from build123d import *

# Parameters (mm, degrees)
SKETCH1_W                = 37
SKETCH1_H                = 30
SKETCH1_W_2              = 20
SKETCH1_H_2              = 20
M4_CLEARANCE_HOLE1_D     = 4.5
M4_CLEARANCE_HOLE1_DEPTH = 30
M4_CLEARANCE_HOLE2_D     = 4.5


with BuildPart() as part:
    # Sweep1: sweep along a path in Sketch2
    with BuildLine(Plane.XY) as sweep1_path:
        Line((0, 0), (75, 0))
        ThreePointArc((75, 0), (115, 40), (75, 80))
        Line((75, 80), (-100, 80))
    # Sketch1 → Sweep1 (sweep)
    with BuildSketch(Plane(origin=(0, 0, 0), x_dir=(0, 0, -1), z_dir=(1, 0, 0))):
        Rectangle(SKETCH1_W, SKETCH1_H)
        Rectangle(SKETCH1_W_2, SKETCH1_H_2, mode=Mode.SUBTRACT)
    sweep(path=sweep1_path.line)

    # M4 Clearance Hole1
    with Locations(Plane(origin=(0, 15, 0), x_dir=(1, 0, 0), z_dir=(0, 1, 0))):
        with Locations((8.5, 14.5), (8.5, -14.5)):
            Hole(M4_CLEARANCE_HOLE1_D / 2, depth=M4_CLEARANCE_HOLE1_DEPTH)

    # M4 Clearance Hole2 (through all)
    with Locations(Plane(origin=(0, 95, 0), x_dir=(1, 0, 0), z_dir=(0, 1, 0))):
        with Locations((-91.5, -14.5), (-91.5, 14.5)):
            Hole(M4_CLEARANCE_HOLE2_D / 2)


solid = part.part
Verification items for the finished model (mm, model axes). A direction names the side the tool comes from. Coordinates: 2 decimals unless noted, no trailing zeros. Order: outer loops, then holes, each group sorted by start corner. A loop starts at its lowest first (then second) coordinate and runs counter-clockwise, first axis right, second up. Notation, with made-up numbers: M -12,83 L 0,83 A24 cw 0,95 Z; hole C -34,-7 d3. An arc over 180 degrees is marked long. Return JSON: item names as keys, results as strings.
1) Access from +Z, -Z, +X, -X, +Y, -Y to the whole of each face (thin tool, end or side, straight path). Record for faces 5 (the cylindrical face through (10.286, -0.21, -13.131)), 6 (the flat face through (-14, 65, 0)), 7 (the flat face through (38, 73, 10)), 8 (the flat face through (38, 10, 0)).
Answer list:
{"face 5": "-Y", "face 6": "+Z, -Z, -X", "face 7": "none", "face 8": "-X"}
2) Thickness scan on L1, parallel to Y at x = 41.5, z = 8; L2, parallel to Z at x = 8, y = -3; L3, parallel to Z at x = 104, y = 59.5. Record the ranges inside material, lowest first. Write a range as [from, to].
Answer list:
{"L1": "[-15, -10], [10, 15], [65, 70], [90, 95]", "L2": "[-18.5, -16.69], [-12.31, -10], [10, 12.31], [16.69, 18.5]", "L3": "[-18.5, -10], [10, 18.5]"}
3) Cross-section at B-B, the plane z = 14.5. Record the boundary of the cut face in (x, y).
Answer list:
{"outline": "M -100,65 L -93.75,65 L -93.75,95 L -100,95 Z; M -89.25,65 L 75,65 A25 cw 75,15 L 10.75,15 L 10.75,-15 L 75,-15 A55 ccw 75,95 L -89.25,95 Z; M 0,-15 L 6.25,-15 L 6.25,15 L 0,15 Z"}
4) Cross-section at C-C, the plane x = 8.5. Record the boundary of the cut face in (y, z).
Answer list:
{"outline": "M -15,-18.5 L 15,-18.5 L 15,-16.75 L -15,-16.75 Z; M -15,-12.25 L 15,-12.25 L 15,12.25 L -15,12.25 Z; M -15,16.75 L 15,16.75 L 15,18.5 L -15,18.5 Z; M 65,-18.5 L 95,-18.5 L 95,18.5 L 65,18.5 Z; hole M -10,-10 L 10,-10 L 10,10 L -10,10 Z; hole M 70,-10 L 90,-10 L 90,10 L 70,10 Z"}
5) Cross-section at D-D, the plane z = -3.5. Record the boundary of the cut face in (x, y).
Answer list:
{"outline": "M -100,65 L 75,65 A25 cw 75,15 L 0,15 L 0,10 L 75,10 A30 ccw 75,70 L -100,70 Z; M -100,90 L 75,90 A50 cw 75,-10 L 0,-10 L 0,-15 L 75,-15 A55 ccw 75,95 L -100,95 Z"}
6) Release check for a two-part mould opening along Z. For faces 1 (the cylindrical face through (104.993, 39.34, -0.14)), 2 (the flat face through (38, -10, 0)), 3 (the cylindrical face through (129.987, 38.791, -0.259)), 4 (the flat face through (42, 76, -18.5)) record: +Z half, -Z half, draft (parallel to the pull), parting line (faces both ways), or undercut.
Answer list:
{"face 1": "undercut", "face 2": "undercut", "face 3": "draft", "face 4": "-Z half"}
7) Gauge pin test, flat ends, axial feed: pin 1 (8 mm diameter, centred on x = -27.5, z = -10, fed in from -Y); pin 2 (2.5 mm diameter, centred on x = -91.5, z = -14.5, fed in from -Y); pin 3 (1 mm diameter, centred on y = 7.5, z = 8, fed in from -X). Record the tip position at first contact, or that the pin passes through.
Answer list:
{"pin 1": "y = 65", "pin 2": "through", "pin 3": "x = 112.56"}
8) Cross-section at A-A, the plane x = 66. Record the boundary of the cut face in (y, z), and give its area (3 significant figures).
Answer list:
{"outline": "M -15,-18.5 L 15,-18.5 L 15,18.5 L -15,18.5 Z; M 65,-18.5 L 95,-18.5 L 95,18.5 L 65,18.5 Z; hole M -10,-10 L 10,-10 L 10,10 L -10,10 Z; hole M 70,-10 L 90,-10 L 90,10 L 70,10 Z", "area": "1,420 mm2"}
